Study the drawing (mm; zero at the part's minimum x, y, z) and answer. Coordinates: 2 decimals unless noted, no trailing zeros. Loops run counter-clockwise (first coordinate to the right, second up) from the corner with the lowest first, then second, coordinate; pieces in that order, holes last. Notation, with made-up numbers: (87, 89) -> (132, 89) arc R19 ccw to (132, 114) -> close; hole circle Ø11 at (51.25, 41). An arc over 180 degrees is marked (long way). Answer as CSV lines item,"result".
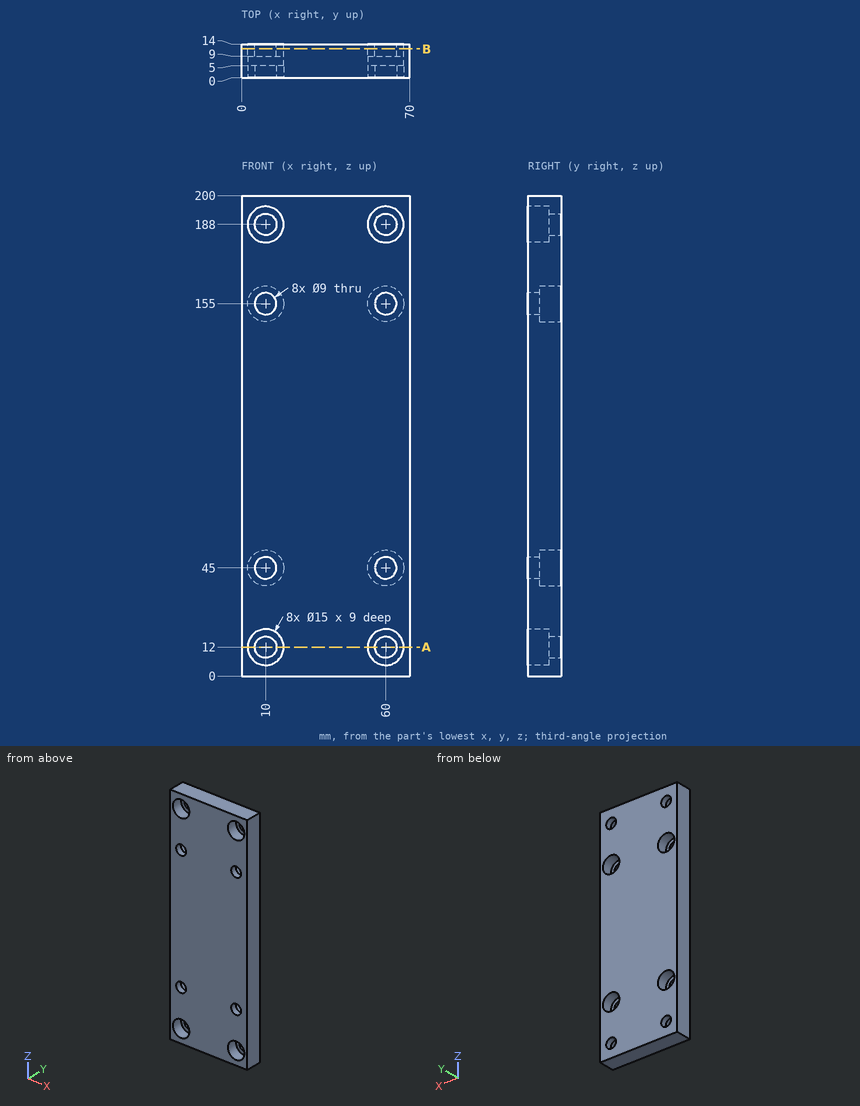
Q1. Find the intervals of material crossed by probe 1 along Z at (x, y) = (10, 11); probe 2 along Z at (x, y) = (10, 3.5); probe 3 along X at (y, z) = (9.75, 45), in increasing order. Write a range as [from, to].
Results:
probe 1,"z = [0, 7.5], [16.5, 37.5], [52.5, 147.5], [162.5, 183.5], [192.5, 200]"
probe 2,"z = [0, 4.5], [19.5, 40.5], [49.5, 150.5], [159.5, 180.5], [195.5, 200]"
probe 3,"x = [0, 2.5], [17.5, 52.5], [67.5, 70]"
Q2. A cutting plane is placed at A-A, the plane z = 12. Write down the section's boundary in (x, y), and give its area (3 significant figures).
Results:
outline,"(0, 0) -> (2.5, 0) -> (2.5, 9) -> (5.5, 9) -> (5.5, 14) -> (0, 14) -> close; (14.5, 9) -> (17.5, 9) -> (17.5, 0) -> (52.5, 0) -> (52.5, 9) -> (55.5, 9) -> (55.5, 14) -> (14.5, 14) -> close; (64.5, 9) -> (67.5, 9) -> (67.5, 0) -> (70, 0) -> (70, 14) -> (64.5, 14) -> close"
area,"620 mm²"
Q3. Given pin 1 Ø7.5 at (x, z) = (7, 186.5) entering from -Y; pin 2 Ø7.5 at (x, z) = (61, 157.5) entering from +Y, each flat-ended and moving along its own axis, determine where each tip first touches the part or whether it passes through.
Results:
pin 1,"stops at y = 9"
pin 2,"stops at y = 5"
Q4. A cutting plane is placed at B-B, the plane y = 12. Give the number of separate pieces and of enclosed holes in the cut face, and give its area (3 significant figures).
Results:
separate pieces,"1"
enclosed holes,"8"
area,"13,000 mm²"
